from build123d import *
from build123d.topology import SkipClean

# Parameters (mm, degrees)
DISC_PROFILE_100_R = 50
DISC_BODY_DEPTH    = 5
FACE_START         = 12
FACE_RIB_1_DEPTH   = 12
FACE_RIB_2_DEPTH   = 12


with BuildPart() as part:
    # Disc Profile Ø100 → Disc Body (new, symmetric)
    with BuildSketch(Plane.XY):
        Circle(DISC_PROFILE_100_R)
    extrude(amount=DISC_BODY_DEPTH, both=True)

    # Face Rib 1 Profile → Face Rib 1 (add)
    with SkipClean():  # the faces are left unmerged after this step: merging them gives an invalid solid
        with BuildSketch(Plane.XY.offset(5).offset(FACE_START)):
            with BuildLine():
                Line((49.638694584, -6), (-49.638694584, -6))
                ThreePointArc((-49.638694584, -6), (-50, 0), (-49.638694584, 6))
                Line((-49.638694584, 6), (49.638694584, 6))
                ThreePointArc((49.638694584, 6), (50, 0), (49.638694584, -6))
            make_face()
        extrude(amount=-FACE_RIB_1_DEPTH)

    # Face Rib 2 Profile → Face Rib 2 (add)
    with SkipClean():  # the faces are left unmerged after this step: merging them gives an invalid solid
        with BuildSketch(Plane(origin=(0, 0, -5), x_dir=(-1, 0, 0), z_dir=(0, 0, -1))):
            with BuildLine():
                Line((-6, -49.638694584), (-6, 49.638694584))
                ThreePointArc((-6, 49.638694584), (0, 50), (6, 49.638694584))
                Line((6, 49.638694584), (6, -49.638694584))
                ThreePointArc((6, -49.638694584), (0, -50), (-6, -49.638694584))
            make_face()
        extrude(amount=FACE_RIB_2_DEPTH)


solid = part.part
Read the model definition and answer for the solid it produces. Units are mm, in the model's axes. A direction names the side the tool comes from. Give positions to 0.01 mm unless a question says otherwise; leave off trailing zeros. Write each loop counter-clockwise with the first axis right and the second up, starting at its lowest first coordinate (ties: lowest second). Pieces come first, ordered by that corner, then holes. Notation, with made-up numbers: (8, 66) - (34, 66) arc R20 cw to (34, 87) - close; hole circle Ø1 at (3, -18.75). An arc over 180 degrees is marked (long way). Use CSV: the item, a comma, the result in double quotes. Start each with the question number.
(1) Determine the mould class of faces 4 (the flat face through (1, -6, 11)), 5 (the flat face through (-1, 6, 11)), 6 (the flat face through (0, 1, -17)) for opening direction Y: +Y half, -Y half, draft (parallel to the pull), parting line (faces both ways), or undercut.
(2) Find section B-B (x = 1). Give the vertices of the cut face in (y, z).
(3) Consider line 1 along Z through (x, y) = (-14, -0.5); line 2 along Z through (x, y) = (-40.5, -11.5); line 3 along X through (y, z) = (2, -10.5). Determine where each line is inside the solid, lowest interval first.
(4) Find section A-A (y = 0). Give the vertices of the cut face in (x, z), plus the area to 3 significant figures.
(5) For faces 1 (the flat face through (-1, -23, 5)), 2 (the flat face through (-1, 23, 5)), 3 (the flat face through (-6, 1, -11)), determine the directions among +Z, -Z, +X, -X, +Y, -Y from which every point of the face is accessible in a straight line to the end or side of a thin tool.
(6) Find section C-C (z = 11). Give the vertices of the cut face in (x, y).
(7) Find section D-D (z = -3). Give the vertices of the cut face in (x, y).
(8) Given P1, Ø2, axis at x = 18.5, z = 3.5, coming from the +Y side; P2, Ø8, axis at y = 24.5, z = 2.5, coming from the +X side; P3, Ø22, axis at x = -38.5, y = 6.5, coming from the -Z side, each flat-ended and moving along its own axis, determine where each tip first touches the part or whether it passes through.
Findings below:
1,face 4,"-Y half"
1,face 5,"+Y half"
1,face 6,"draft"
2,outline,"(-49.99, -17) - (49.99, -17) - (49.99, 5) - (6, 5) - (6, 17) - (-6, 17) - (-6, 5) - (-49.99, 5) - close"
3,line 1,"-5 to 17"
3,line 2,"-5 to 5"
3,line 3,"-6 to 6"
4,outline,"(-50, -5) - (-6, -5) - (-6, -17) - (6, -17) - (6, -5) - (50, -5) - (50, 17) - (-50, 17) - close"
4,area,"2,340 mm2"
5,face 1,"+Z, +X, -X, -Y"
5,face 2,"+Z, +X, -X, +Y"
5,face 3,"-Z, -X, +Y, -Y"
6,outline,"(-49.64, -6) - (49.64, -6) arc R50 ccw to (49.64, 6) - (-49.64, 6) arc R50 ccw to start"
7,outline,"circle Ø100 at (0, 0)"
8,P1,"y = 46.84"
8,P2,"x = 45.6"
8,P3,"z = -5"
